Answer from the drawing. Dimensions are ordinates in mm from the lowest x, y and z of the part. Coordinates: 2 decimals unless noted, no trailing zeros. Order: outer loops, then holes, each group sorted by start corner. A loop starts at its lowest first (then second) coordinate and runs counter-clockwise, first axis right, second up. Notation, with made-up numbers: (43.25, -3.75) -> (85.25, -3.75) arc R29 ccw to (85.25, 23.25) -> close; hole circle Ø5 at (-15, 77). An arc over 180 degrees is marked (long way). Answer as a JSON object with one key per item and string values. Group by question number.
1) Consider L1, parallel to X at y = 2.4, z = 7; L2, parallel to X at y = 4.15, z = 7.5; L3, parallel to Y at x = 23, z = 5.25. Determine where each line is inside the solid, lowest interval first.
2) Section A-A on y = 3 is taken. Determine the outline of the cut face in (x, z).
3) Section C-C on x = 3.25 is taken. Determine the outline of the cut face in (y, z).
4) Section B-B on z = 2.5 is taken. Determine the outline of the cut face in (x, y), and give its area (3 significant figures).
5) Given pin 1 (2 mm diameter, centred on x = 23, y = 3, fed in from -Z), flat-ended and moving along its own axis, determine where the tip first touches the part or whether it passes through.
6) Determine the mould class of the marked faces 1, 2, 3 and 4 for opening direction X: released by +X, released by -X, zero draft, split by the parting line, or undercut.
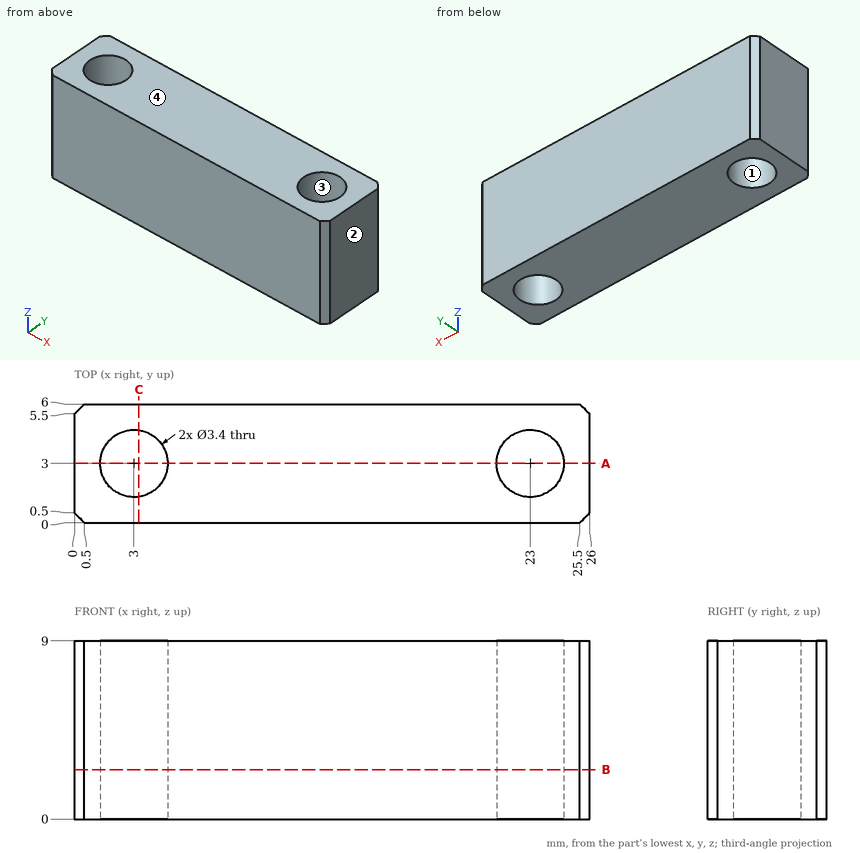
Worked answers:
{
 "1": {"L1": "x = 0 to 1.41, 4.59 to 21.41, 24.59 to 26", "L2": "x = 0 to 1.75, 4.25 to 21.75, 24.25 to 26", "L3": "y = 0 to 1.3, 4.7 to 6"},
 "2": {"outline": "(0, 0) -> (1.3, 0) -> (1.3, 9) -> (0, 9) -> close; (4.7, 0) -> (21.3, 0) -> (21.3, 9) -> (4.7, 9) -> close; (24.7, 0) -> (26, 0) -> (26, 9) -> (24.7, 9) -> close"},
 "3": {"outline": "(0, 0) -> (1.32, 0) -> (1.32, 9) -> (0, 9) -> close; (4.68, 0) -> (6, 0) -> (6, 9) -> (4.68, 9) -> close"},
 "4": {"outline": "(0, 0.5) -> (0.5, 0) -> (25.5, 0) -> (26, 0.5) -> (26, 5.5) -> (25.5, 6) -> (0.5, 6) -> (0, 5.5) -> close; hole circle Ø3.4 at (3, 3); hole circle Ø3.4 at (23, 3)", "area": "137 mm²"},
 "5": {"pin 1": "passes through"},
 "6": {"face 1": "undercut", "face 2": "released by +X", "face 3": "undercut", "face 4": "zero draft"}
}
